Can you work these out from the model? Positions are in its coordinate system, mm. Give positions to 0.01 mm unless a question says otherwise; leave off trailing zeros. Loops run counter-clockwise (first coordinate to the right, second up) from the corner with the lowest first, then second, coordinate; pieces in that order, holes last. Notation, with made-up numbers: (-4, -38) - (47, -38) arc R31 ccw to (47, -1) - close; hole circle Ø3 at (30, 33.25). An arc over 180 degrees is marked (long way). Answer as a JSON object with one key per item and string values. Group by question number.
Item 1: Will these pins go through, and if not, where does the flat tip stop? pin 1 (0.9 mm diameter, centred on y = 208, z = -6, fed in from +X); pin 2 (4.5 mm diameter, centred on x = 16.5, y = 291.5, fed in from -Z); pin 3 (4 mm diameter, centred on y = 217, z = 10, fed in from -X).
Item 2: Suppose I cut it at B-B on z = 0. Write out the boundary of the cut face in (x, y), and give its area (3 significant figures).
Item 3: Thinking about a two-plate mould opening in Z: for faces 1 (the cylindrical face through (17.5, 277.6, -0.1)), 2 (the flat face through (0, 278, -8)), 3 (the flat face through (0, 278, 17)), which applies, pulls with the +Z half, pulls with the -Z half, needs draft (parallel to the pull), parting line crosses it, or undercut?
Item 4: Please list where these lines run through material, in increasing order: L1, parallel to X at y = 278, z = -5.5; L2, parallel to X at y = 484.5, z = -0.5; L3, parallel to Z at x = -16, y = 530.
Item 5: Suppose I cut it at A-A on y = 349.5. Write out the boundary of the cut face in (x, z).
from build123d import *

# Parameters (mm, degrees)
EXTRUDE_1_DEPTH = 563


with BuildPart() as part:
    # 草图1 → 凸台-拉伸1 (new body)
    with BuildSketch(Plane(origin=(0, 0, 0), x_dir=(1, 0, 0), z_dir=(0, 1, 0))):
        with BuildLine():
            Line((-12.5, 5), (-12.5, 8))
            Line((-12.5, 8), (12.5, 8))
            Line((12.5, 8), (12.5, 5))
            ThreePointArc((12.5, 5), (17.5, 0), (12.5, -5))
            Line((12.5, -5), (12.5, -13))
            Line((12.5, -13), (18, -13))
            Line((18, -13), (18, -17))
            Line((18, -17), (-18, -17))
            Line((-18, -17), (-18, -13))
            Line((-18, -13), (-12.5, -13))
            Line((-12.5, -13), (-12.5, -5))
            ThreePointArc((-12.5, -5), (-17.5, 0), (-12.5, 5))
        make_face()
    extrude(amount=EXTRUDE_1_DEPTH)


solid = part.part
Worked out:
{
 "1": {"pin 1": "stops at x = 12.5", "pin 2": "stops at z = -4.68", "pin 3": "stops at x = -12.5"},
 "2": {"outline": "(-17.5, 0) - (17.5, 0) - (17.5, 563) - (-17.5, 563) - close", "area": "19,700 mm2"},
 "3": {"face 1": "undercut", "face 2": "pulls with the -Z half", "face 3": "pulls with the +Z half"},
 "4": {"L1": "x = -12.5 to 12.5", "L2": "x = -17.47 to 17.47", "L3": "z = -3.57 to 3.57, 13 to 17"},
 "5": {"outline": "(-18, 13) - (-12.5, 13) - (-12.5, 5) arc R5 ccw to (-12.5, -5) - (-12.5, -8) - (12.5, -8) - (12.5, -5) arc R5 ccw to (12.5, 5) - (12.5, 13) - (18, 13) - (18, 17) - (-18, 17) - close"}
}
